Can you work these out from the drawing? Everything is in mm from the part's minimum corner. A direction names the side the tool comes from. Give positions to 0.01 mm unless a question says otherwise; leave off trailing zeros. Order: outer loops, then holes, each group sorted by start corner. A loop starts at its lowest first (then second) coordinate and runs counter-clockwise, first axis right, second up. Notation, with made-up numbers: (-2.5, -3.5) -> (46.5, -3.5) arc R23 ccw to (46.5, 10.5) -> close; hole circle Ø3 at (84, 86). An arc over 180 degrees is marked (long way). Answer as CSV lines item,"result". Start each with the question number.
(1) I want a section at C-C (y = 21). Please give me the cut outline in (x, z), plus the area to 3 significant figures.
(2) On a 3-axis mill with a long thin cutter (end or side, diameter ignored), from which of +Z, -Z, +X, -X, +Y, -Y can I reach the whole of each face in a straight line? I mean the marked faces 5, 6, 7 and 8. Say none if no direction works.
(3) I want a section at D-D (z = 15). Please give me the cut outline in (x, y), plus the area to 3 significant figures.
(4) Will these pins go through, and if not, where does the flat tip stop? pin 1 Ø11 at (x, z) = (18, 16) entering from +Y; pin 2 Ø6 at (y, z) = (32, 11) entering from +X; pin 3 Ø12 at (y, z) = (25, 12) entering from -X.
(5) We'd pull the mould along Y, two halves only. Please class the marked faces 1, 2, 3 and 4: released by +Y, released by -Y, zero draft, split by the parting line, or undercut.
(6) I want a section at B-B (z = 3.5). Please give me the cut outline in (x, y), plus the area to 3 significant figures.
(7) I need wall thicknesses on L1, parallel to Z at x = 61, y = 21; L2, parallel to Y at x = 3, z = 29; L3, parallel to X at y = 4, z = 25.5. Which ranges of each line are inside material? Lowest first, please.
(8) I want a section at A-A (x = 40). Please give me the cut outline in (y, z).
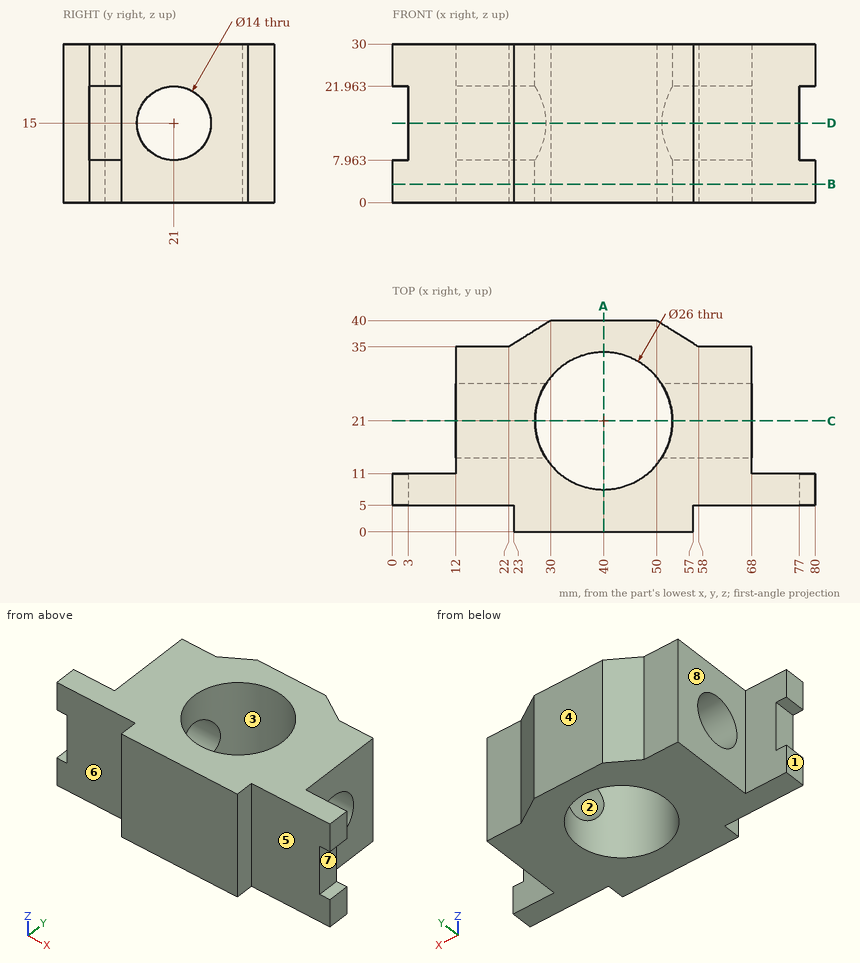
Final values:
1,outline,"(12, 0) -> (27, 0) -> (27, 8) -> (12, 8) -> close; (12, 22) -> (27, 22) -> (27, 30) -> (12, 30) -> close; (53, 0) -> (68, 0) -> (68, 8) -> (53, 8) -> close; (53, 22) -> (68, 22) -> (68, 30) -> (53, 30) -> close"
1,area,"480 mm²"
2,face 5,"+Z, -Z, +X, -Y"
2,face 6,"+Z, -Z, -X, -Y"
2,face 7,"+X, +Y, -Y"
2,face 8,"+Z, -Z, -X, +Y"
3,outline,"(3, 5) -> (23, 5) -> (23, 0) -> (57, 0) -> (57, 5) -> (77, 5) -> (77, 11) -> (68, 11) -> (68, 14) -> (50.95, 14) arc R13 cw to (29.05, 14) -> (12, 14) -> (12, 11) -> (3, 11) -> close; (12, 28) -> (29.05, 28) arc R13 cw to (50.95, 28) -> (68, 28) -> (68, 35) -> (58, 35) -> (50, 40) -> (30, 40) -> (22, 35) -> (12, 35) -> close"
3,area,"1,130 mm²"
4,pin 1,"y = 35.94"
4,pin 2,"x = 68"
4,pin 3,"x = 12"
5,face 1,"zero draft"
5,face 2,"undercut"
5,face 3,"undercut"
5,face 4,"released by +Y"
6,outline,"(0, 5) -> (23, 5) -> (23, 0) -> (57, 0) -> (57, 5) -> (80, 5) -> (80, 11) -> (68, 11) -> (68, 35) -> (58, 35) -> (50, 40) -> (30, 40) -> (22, 35) -> (12, 35) -> (12, 11) -> (0, 11) -> close; hole circle Ø26 at (40, 21)"
6,area,"1,600 mm²"
7,L1,"0 to 8, 22 to 30"
7,L2,"5 to 11"
7,L3,"23 to 57"
8,outline,"(0, 0) -> (8, 0) -> (8, 30) -> (0, 30) -> close; (34, 0) -> (40, 0) -> (40, 30) -> (34, 30) -> close"
